```python
from build123d import *

# Parameters (mm, degrees)
SKETCH1_R           = 5
BOSS_EXTRUDE1_DEPTH = 4.5


with BuildPart() as part:
    # Sketch1 → Boss-Extrude1 (new body)
    with BuildSketch(Plane(origin=(0, 0, 0), x_dir=(1, 0, 0), z_dir=(0, 1, 0))):
        with BuildLine():
            Line((0, 0), (271.5, 0))
            ThreePointArc((271.5, 0), (275.035533906, -1.464466094), (276.5, -5))
            Line((276.5, -5), (276.5, -45))
            ThreePointArc((276.5, -45), (277.964466094, -48.535533906), (281.5, -50))
            Line((281.5, -50), (628.5, -50))
            Line((628.5, -50), (628.5, -72))
            Line((628.5, -72), (251.5, -72))
            ThreePointArc((251.5, -72), (247.964466094, -70.535533906), (246.5, -67))
            Line((246.5, -67), (246.5, -27))
            ThreePointArc((246.5, -27), (245.035533906, -23.464466094), (241.5, -22))
            Line((241.5, -22), (121.33715964, -22))
            ThreePointArc((121.33715964, -22), (114.86759563, -20.924712455), (109.09369578, -17.814474152))
            Line((109.09369578, -17.814474152), (104.40630422, -14.185525848))
            ThreePointArc((104.40630422, -14.185525848), (98.63240437, -11.075287545), (92.16284036, -10))
            Line((92.16284036, -10), (80.83715964, -10))
            ThreePointArc((80.83715964, -10), (74.36759563, -11.075287545), (68.59369578, -14.185525848))
            Line((68.59369578, -14.185525848), (63.90630422, -17.814474152))
            ThreePointArc((63.90630422, -17.814474152), (58.13240437, -20.924712455), (51.66284036, -22))
            Line((51.66284036, -22), (0, -22))
            Line((0, -22), (0, 0))
        make_face()
        with Locations(Location((618.5, -60, 0), (0, 0, 270))):
            Circle(SKETCH1_R, mode=Mode.SUBTRACT)
    extrude(amount=BOSS_EXTRUDE1_DEPTH)


solid = part.part
```
Design review of the part built by this model. Coordinates are the model's own, in mm. Give positions to 0.01 mm unless a question says otherwise; leave off trailing zeros. Loops run counter-clockwise (first coordinate to the right, second up) from the corner with the lowest first, then second, coordinate; pieces in that order, holes last. Notation, with made-up numbers: (-0.5, 57) -> (57.5, 57) arc R17 cw to (57.5, 83) -> close; hole circle Ø1 at (-27.75, 38.5). An arc over 180 degrees is marked (long way). Write each question's results on one line, items separated by ' | '.
Q1. Take a section at B-B, the plane x = 449.5. Write out the cut boundary in (y, z).
Reply:
outline: (0, 50) -> (4.5, 50) -> (4.5, 72) -> (0, 72) -> close
Q2. The part is to be moulded in two halves that separate along X. For faces 1 (the face through (319, 0, 51)), 2 (the face through (614.064, 2.218, 62.307)), say which applies: +X half, -X half, draft (parallel to the pull), parting line (faces both ways), or undercut.
Reply:
face 1: draft | face 2: undercut
Q3. For pin 1 Ø9 at (x, z) = (618.5, 60) entering from +Y; pin 2 Ø1 at (y, z) = (0.5, 20.5) entering from +X; pin 3 Ø1.3 at (x, y) = (157.5, 2.5) entering from +Z; pin 4 Ø1.3 at (x, y) = (86.5, 2) entering from +Z, all flat-tipped, find the tip position at first contact; note any pin that passes through.
Reply:
pin 1: passes through | pin 2: stops at x = 276.5 | pin 3: stops at z = 22 | pin 4: stops at z = 10
Q4. Take a section at A-A, the plane y = 2.65. Write out the cut boundary in (x, z).
Reply:
outline: (0, 0) -> (271.5, 0) arc R5 ccw to (276.5, 5) -> (276.5, 45) arc R5 cw to (281.5, 50) -> (628.5, 50) -> (628.5, 72) -> (251.5, 72) arc R5 ccw to (246.5, 67) -> (246.5, 27) arc R5 cw to (241.5, 22) -> (121.34, 22) arc R20 ccw to (109.09, 17.81) -> (104.41, 14.19) arc R20 cw to (92.16, 10) -> (80.84, 10) arc R20 cw to (68.59, 14.19) -> (63.91, 17.81) arc R20 ccw to (51.66, 22) -> (0, 22) -> close; hole circle Ø10 at (618.5, 60)
Q5. Wall thickness on L1, parallel to Z at x = 618.5, y = 2.35; L2, parallel to X at y = 1.9, z = 60; L3, parallel to X at y = 2.05, z = 44: over which ranges is each line inside the solid? List them lowest first.
Reply:
L1: z = 50 to 55, 65 to 72 | L2: x = 246.5 to 613.5, 623.5 to 628.5 | L3: x = 246.5 to 276.5
